Check sheet for the modelled part. Datum: model origin and axes. Units: mm. Give positions to 0.01 mm unless a question says otherwise; leave off trailing zeros. Write each loop counter-clockwise with the first axis right and the second up, starting at its lowest first coordinate (ties: lowest second). Pieces come first, ordered by that corner, then holes. Notation, with made-up numbers: (-24, 48) - (-18, 48) arc R18 cw to (-18, 52) - close; hole circle Ø4 at (69, 34). An arc over 180 degrees is marked (long way). Return JSON: item names as keys, results as strings. Group by question number.
```python
from build123d import *

# Parameters (mm, degrees)
EXTRUDE_1_DEPTH     = 700
SKETCH_2_W          = 750
SKETCH_2_H          = 1200
CUT_EXTRUDE_1_DEPTH = 43
SKETCH_3_W          = 754
SKETCH_3_H          = 1204
SKETCH_3_W_2        = 750
SKETCH_3_H_2        = 1200
EXTRUDE_2_DEPTH     = 24
EXTRUDE_3_DEPTH     = 2
EXTRUDE_4_DEPTH     = 2
SKETCH_6_W          = 980
SKETCH_6_H          = 30
EXTRUDE_5_DEPTH     = 2
EXTRUDE_7_DEPTH     = 2
SKETCH_9_R          = 4.5
CUT_EXTRUDE_2_DEPTH = 10
CUT_EXTRUDE_3_DEPTH = 45
SKETCH_11_R         = 4.5
CUT_EXTRUDE_4_DEPTH = 5
SKETCH_12_R         = 4.5
CUT_EXTRUDE_5_DEPTH = 10


with BuildPart() as part:
    # Sketch 1 → Extrude 1 (new, symmetric)
    with BuildSketch(Plane.XY):
        Polygon((490, 0), (460, 0), (460, 2), (488, 2), (488, 98), (-389.171572875, 98), (-485.171572875, 2), (-460, 2), (-460, 0), (-490, 0), (-390, 100), (490, 100), align=None)
    extrude(amount=EXTRUDE_1_DEPTH, both=True)

    # Sketch 2 → Cut-Extrude 1 (cut)
    with BuildSketch(Plane(origin=(0, 100, 0), x_dir=(1, 0, 0), z_dir=(0, 1, 0))):
        with Locations((50, 0)):
            Rectangle(SKETCH_2_W, SKETCH_2_H)
    extrude(amount=-CUT_EXTRUDE_1_DEPTH, mode=Mode.SUBTRACT)

    # Sketch 3 → Extrude 2 (add)
    with BuildSketch(Plane(origin=(0, 100, 0), x_dir=(1, 0, 0), z_dir=(0, 1, 0))):
        with Locations((50, 0)):
            Rectangle(SKETCH_3_W, SKETCH_3_H)
        with Locations((50, 0)):
            Rectangle(SKETCH_3_W_2, SKETCH_3_H_2, mode=Mode.SUBTRACT)
    extrude(amount=-EXTRUDE_2_DEPTH)

    # Sketch 4 → Extrude 3 (add)
    with BuildSketch(Plane.XZ.offset(-76)):
        Polygon((-327, 602), (427, 602), (427, 572), (427, -572), (427, -602), (-327, -602), (-327, -572), (397, -572), (397, 0), (397, 572), (-327, 572), align=None)
    extrude(amount=-EXTRUDE_3_DEPTH)



with BuildPart() as body_2:
    # Sketch 5 → Extrude 4 (new body)
    with BuildSketch(Plane(origin=(0, 0, -700), x_dir=(-1, 0, 0), z_dir=(0, 0, -1))):
        Polygon((-490, 100), (-490, 0), (490, 0), (390, 100), align=None)
    extrude(amount=-EXTRUDE_4_DEPTH)


with BuildPart() as part_1:
    add(part.part)

    add(body_2.part)  # Extrude 5 merges body 2
    # Sketch 6 → Extrude 5 (add)
    with BuildSketch(Plane.XZ):
        with Locations((0, -685)):
            Rectangle(SKETCH_6_W, SKETCH_6_H)
    extrude(amount=-EXTRUDE_5_DEPTH)

    # Sketch 8 → Extrude 7 (add)
    with BuildSketch(Plane.XY.offset(700)):
        Polygon((490, 0), (490, 100), (-390, 100), (-490, 0), (-460, 0), (460, 0), align=None)
    extrude(amount=-EXTRUDE_7_DEPTH)

    # Sketch 9 → Cut-Extrude 2 (cut)
    with BuildSketch(Plane(origin=(0, 0, 698), x_dir=(-1, 0, 0), z_dir=(0, 0, -1))):
        with Locations((-460, 84)):
            Circle(SKETCH_9_R)
        with Locations((250, 84)):
            Circle(SKETCH_9_R)
        with Locations((190, 84)):
            Circle(SKETCH_9_R)
        with Locations((447.012193309, 20.360389693)):
            Circle(SKETCH_9_R)
        with Locations((-100, 84)):
            Circle(SKETCH_9_R)
    extrude(amount=-CUT_EXTRUDE_2_DEPTH, mode=Mode.SUBTRACT)

    # Sketch 10 → Cut-Extrude 3 (cut)
    with BuildSketch(Plane(origin=(0, 0, -700), x_dir=(-1, 0, 0), z_dir=(0, 0, -1))):
        Polygon((478.109799219, 11.890200781), (488, 2), (495.020614582, -5.020614582), (488.781283968, 5.695100391), align=None)
    extrude(amount=-CUT_EXTRUDE_3_DEPTH, mode=Mode.SUBTRACT)

    # Sketch 11 → Cut-Extrude 4 (cut)
    with BuildSketch(Plane.XZ):
        with Locations((-474, 670)):
            Circle(SKETCH_11_R)
        with Locations((-474, 0)):
            Circle(SKETCH_11_R)
        with Locations((-474, -684)):
            Circle(SKETCH_11_R)
        with Locations((0, -684)):
            Circle(SKETCH_11_R)
        with Locations(Location((474, -684, 0), (0, 0, 270))):
            Circle(SKETCH_11_R)
        with Locations(Location((474, 0, 0), (0, 0, 270))):
            Circle(SKETCH_11_R)
        with Locations(Location((474, 670, 0), (0, 0, 270))):
            Circle(SKETCH_11_R)
    extrude(amount=-CUT_EXTRUDE_4_DEPTH, mode=Mode.SUBTRACT)

    # Sketch 12 → Cut-Extrude 5 (cut)
    with BuildSketch(Plane.ZY.offset(-488)):
        with Locations((670, 70)):
            Circle(SKETCH_12_R)
        with Locations((330, 70)):
            Circle(SKETCH_12_R)
    extrude(amount=-CUT_EXTRUDE_5_DEPTH, mode=Mode.SUBTRACT)


solid = part_1.part
```
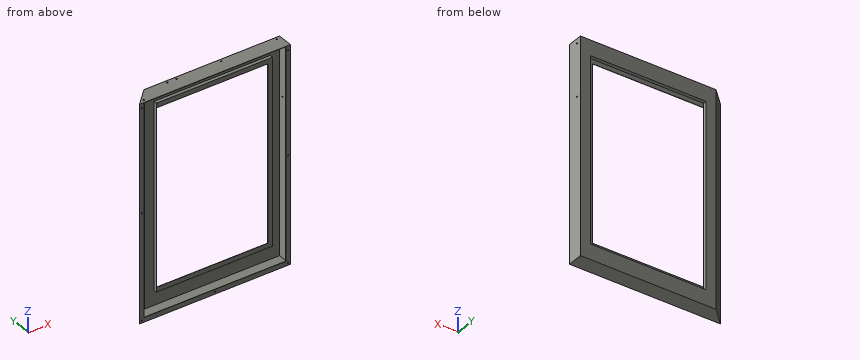
Item 1: Depth check by flat-ended pin: pin 1 (8 mm diameter, centred on x = -474, z = 0, fed in from -Y); pin 2 (14.5 mm diameter, centred on y = 70, z = 330, fed in from -X); pin 3 (0.6 mm diameter, centred on y = 1.5, z = -310, fed in from -X). Enter the tip coordinate at first touch or a pass-through.
Item 2: Material ranges on line 1 along Z through (x, y) = (474, 1.45); line 2 along Z through (x, y) = (333.5, 33.5); line 3 along Z through (x, y) = (-85, 85), recorded low to high. Write a range as from..to.
Item 3: Section check B-B on z = -133. Record the cut outline in (x, y), plus the area to 3 significant figures.
Item 4: Section check A-A on x = -122. Record the cut outline in (y, z), plus the area to 3 significant figures.
Reply:
{
 "1": {"pin 1": "y = 9.17", "pin 2": "x = -427.25", "pin 3": "x = -488.8"},
 "2": {"line 1": "-700..-688.5, -679.5..-4.5, 4.5..665.5, 674.5..700", "line 2": "-700..-698, 698..700", "line 3": "-700..-698, -602..-600, 600..602, 698..700"},
 "3": {"outline": "(-490, 0) - (-460, 0) - (-460, 2) - (-485.17, 2) - (-389.17, 98) - (-327, 98) - (-327, 76) - (-325, 76) - (-325, 100) - (-390, 100) - close; (397, 76) - (427, 76) - (427, 98) - (488, 98) - (488, 2) - (460, 2) - (460, 0) - (490, 0) - (490, 100) - (425, 100) - (425, 78) - (397, 78) - close", "area": "988 mm²"},
 "4": {"outline": "(0, -700) - (100, -700) - (100, -600) - (78, -600) - (78, -572) - (76, -572) - (76, -602) - (98, -602) - (98, -698) - (2, -698) - (2, -670) - (0, -670) - close; (0, 698) - (98, 698) - (98, 602) - (76, 602) - (76, 572) - (78, 572) - (78, 600) - (100, 600) - (100, 700) - (0, 700) - close", "area": "1,050 mm²"}
}
